For this review, take the finished solid that the model builds, in its own axes (mm). Coordinates: 2 decimals unless noted, no trailing zeros. Order: outer loops, then holes, each group sorted by start corner. A loop starts at its lowest first (then second) coordinate and runs counter-clockwise, first axis right, second up. Notation, with made-up numbers: (42, -10) -> (73, -10) arc R26 ccw to (73, 21) -> close; hole circle Ø2 at (18, 19). An arc over 180 degrees is marked (long way). Return JSON: item names as keys, results as strings. Group by question number.
Item 1: Take a section at C-C (x = -3). Write out the cut boundary in (y, z), then the cut area to 3 significant figures.
Item 2: Take a section at B-B (y = 24.5). Write out the cut boundary in (x, z), then the cut area to 3 significant figures.
Item 3: Take a section at A-A (z = 469.5). Write out the cut boundary in (x, y).
Item 4: Insertion check: pin 1 (4 mm diameter, centred on x = 15, z = -556.5, fed in from +Y); pin 2 (8 mm diameter, centred on x = 4.5, z = -395.5, fed in from +Y). Each pin has a flat end and moves straight along its axis. Give the tip position at first contact, or say it passes through.
Item 5: For line 1 along X through (y, z) = (30, 777); line 2 along X through (y, z) = (31, -260.5); line 3 along Y through (x, z) = (4, -739), list the stretches that pass through material, from the lowest coordinate up.
```python
from build123d import *

# Parameters (mm, degrees)
EXTRUDE1_DEPTH = 1000


with BuildPart() as part:
    # Sketch1 → Extrude1 (new, symmetric)
    with BuildSketch(Plane.XY):
        with BuildLine():
            Line((-25, 0), (25, 0))
            Line((25, 0), (25, 37))
            ThreePointArc((25, 37), (22.671841203, 36.084021126), (21.549999087, 33.847771823))
            Line((21.549999087, 33.847771823), (19.250000913, 10.804761752))
            ThreePointArc((19.250000913, 10.804761752), (16.982128941, 6.310266493), (12.284611923, 4.5))
            Line((12.284611923, 4.5), (-12.284611923, 4.5))
            ThreePointArc((-12.284611923, 4.5), (-16.982128941, 6.310266493), (-19.250000913, 10.804761752))
            Line((-19.250000913, 10.804761752), (-21.549999087, 33.847771823))
            ThreePointArc((-21.549999087, 33.847771823), (-22.671841203, 36.084021126), (-25, 37))
            Line((-25, 37), (-25, 0))
        make_face()
    extrude(amount=EXTRUDE1_DEPTH, both=True)


solid = part.part
```
Findings below:
{
 "1": {"outline": "(0, -1000) -> (4.5, -1000) -> (4.5, 1000) -> (0, 1000) -> close", "area": "9,000 mm2"},
 "2": {"outline": "(-25, -1000) -> (-20.62, -1000) -> (-20.62, 1000) -> (-25, 1000) -> close; (20.62, -1000) -> (25, -1000) -> (25, 1000) -> (20.62, 1000) -> close", "area": "17,500 mm2"},
 "3": {"outline": "(-25, 0) -> (25, 0) -> (25, 37) arc R3.5 ccw to (21.55, 33.85) -> (19.25, 10.8) arc R7 cw to (12.28, 4.5) -> (-12.28, 4.5) arc R7 cw to (-19.25, 10.8) -> (-21.55, 33.85) arc R3.5 ccw to (-25, 37) -> close"},
 "4": {"pin 1": "stops at y = 6.33", "pin 2": "stops at y = 4.5"},
 "5": {"line 1": "x = -25 to -21.17, 21.17 to 25", "line 2": "x = -25 to -21.27, 21.27 to 25", "line 3": "y = 0 to 4.5"}
}
